The drawing under review shows one solid part. Ordinate dimensions are in mm from its lowest x, y, z. Coordinates: 2 decimals unless noted, no trailing zeros. Order: outer loops, then holes, each group sorted by start corner. A loop starts at its lowest first (then second) coordinate and runs counter-clockwise, first axis right, second up. Notation, with made-up numbers: (35.5, -40) -> (46.5, -40) arc R7 cw to (46.5, -32) -> close; hole circle Ø8 at (4, 88). An arc over 180 degrees is marked (long way). Use one line per item in the form item = value.
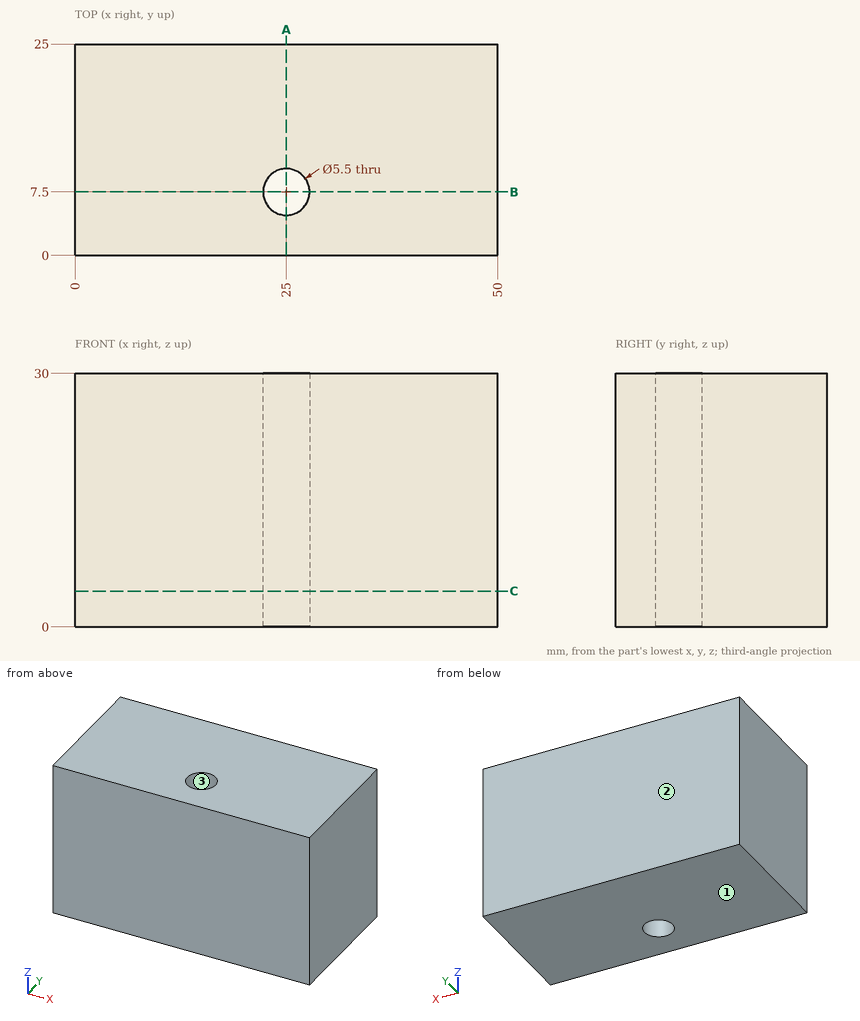
Item 1: Draft analysis for pull direction Y (two halves, no side actions). For the marked faces 1, 2 and 3, state which applies: released by +Y, released by -Y, zero draft, split by the parting line, or undercut.
Results found:
face_1 = zero draft
face_2 = released by +Y
face_3 = undercut
Item 2: To check wall thickness, follow L1, parallel to Y at x = 25, z = 10.75; L2, parallel to X at y = 5, z = 12.5; L3, parallel to X at y = 6.5, z = 1.5. State the ranges of each line that lie inside material, in increasing order. Write a range as from..to.
Results found:
L1 = 0..4.75, 10.25..25
L2 = 0..23.85, 26.15..50
L3 = 0..22.44, 27.56..50
Item 3: We need section A-A (x = 25). Write out the cut boundary in (y, z), plus the area to 3 significant figures.
Results found:
outline = (0, 0) -> (4.75, 0) -> (4.75, 30) -> (0, 30) -> close; (10.25, 0) -> (25, 0) -> (25, 30) -> (10.25, 30) -> close
area = 585 mm²
Item 4: We need section C-C (z = 4.25). Write out the cut boundary in (x, y).
Results found:
outline = (0, 0) -> (50, 0) -> (50, 25) -> (0, 25) -> close; hole circle Ø5.5 at (25, 7.5)
Item 5: We need section B-B (y = 7.5). Write out the cut boundary in (x, z).
Results found:
outline = (0, 0) -> (22.25, 0) -> (22.25, 30) -> (0, 30) -> close; (27.75, 0) -> (50, 0) -> (50, 30) -> (27.75, 30) -> close
